Part model, mm, in its own coordinate system. Face numbers are marked on the shaded views. Give positions to 0.01 mm unless a question says otherwise; leave off trailing zeros. Order: outer loops, then holes, each group sorted by start corner. A loop starts at its lowest first (then second) coordinate and runs counter-clockwise, first axis right, second up.
1. Slice it at A-A on z = 4. List the corners of the cut face in (x, y).
2. Probe line 1 (Y direction, x = -8.5, z = 3); line 2 (Y direction, x = 3.5, z = 7.75); line 3 (X direction, y = 4, z = 9). List the from-to ranges inside material, lowest first.
3. Slice it at C-C on x = 0. List the corners of the cut face in (y, z), and give its area (3 significant figures).
4. Slice it at D-D on y = 12. List the corners of the cut face in (x, z).
5. Mould opens along X. For the marked faces 1, 2 and 3 say: +X half, -X half, draft (parallel to the pull), parting line (faces both ways), or undercut.
6. Slice it at B-B on y = -7.25. List the corners of the cut face in (x, z), and give its area (3 significant figures).
7. Drop flat-ended pins along their axis: pin 1 Ø2 at (x, z) = (-3, 6) entering from -Y; pin 2 Ø2 at (y, z) = (-2.5, 9) entering from -X; pin 3 Ø1 at (y, z) = (7, 3.5) entering from -X. Give the stop position or say it passes through.
from build123d import *

# Parameters (mm, degrees)
SKETCH1_R           = 10
BOSS_EXTRUDE1_DEPTH = 10


with BuildPart() as part:
    # Sketch1 → Boss-Extrude1 (new body)
    with BuildSketch(Plane.XY):
        Polygon((10.724675699, 9.659951577), (-3.003425616, 14.117817392), (-13.728101315, 4.457865814), (-10.724675699, -9.659951577), (3.003425616, -14.117817392), (13.728101315, -4.457865814), align=None)
        Circle(SKETCH1_R, mode=Mode.SUBTRACT)
    extrude(amount=BOSS_EXTRUDE1_DEPTH)


solid = part.part
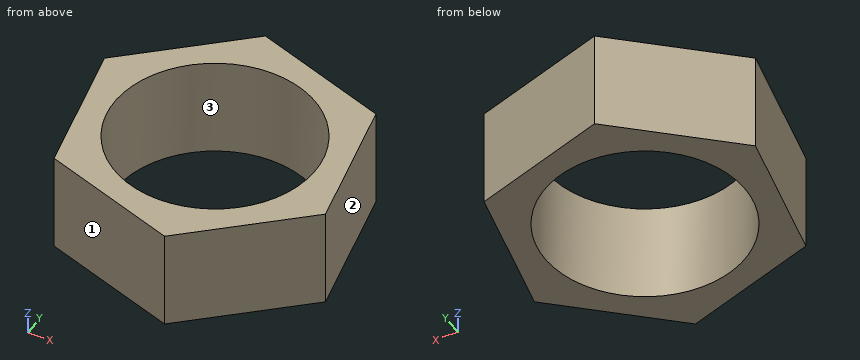
Data:
1. outline: (-13.73, 4.46) - (-10.72, -9.66) - (3, -14.12) - (13.73, -4.46) - (10.72, 9.66) - (-3, 14.12) - close; hole circle Ø20 at (0, 0)
2. line 1: y = -10.38 to -5.27, 5.27 to 9.17
2. line 2: y = -13.67 to -9.37, 9.37 to 12.01
2. line 3: x = -13.63 to -9.17, 9.17 to 11.93
3. outline: (-13.14, 0) - (-10, 0) - (-10, 10) - (-13.14, 10) - close; (10, 0) - (13.14, 0) - (13.14, 10) - (10, 10) - close
3. area: 62.9 mm2
4. outline: (-5.35, 0) - (3.52, 0) - (3.52, 10) - (-5.35, 10) - close
5. face 1: -X half
5. face 2: +X half
5. face 3: undercut
6. outline: (-11.24, 0) - (-6.89, 0) - (-6.89, 10) - (-11.24, 10) - close; (6.89, 0) - (10.63, 0) - (10.63, 10) - (6.89, 10) - close
6. area: 80.9 mm2
7. pin 1: stops at y = -12.49
7. pin 2: stops at x = -12.46
7. pin 3: stops at x = -11.46
